Build history of the part. All positions in model axes, mm. Face numbers are marked on the shaded views. Give positions to 0.01 mm unless a question says otherwise; leave off trailing zeros. Loops run counter-clockwise (first coordinate to the right, second up) from the corner with the lowest first, then second, coordinate; pieces in that order, holes last. Notation, with made-up numbers: M 42.5,-13.5 L 77.5,-13.5 A28 ccw 77.5,15.5 Z; hole C 62.25,36.5 d9. An arc over 180 degrees is marked long. Answer in a Markdown table with one row per item. Add a question column.
```python
from build123d import *

# Parameters (mm, degrees)
SKETCH1_R           = 7
BOSS_EXTRUDE1_DEPTH = 10


with BuildPart() as part:
    # Sketch1 → Boss-Extrude1 (new body)
    with BuildSketch(Plane.XY):
        Polygon((-80, 104), (-30, 17.397459622), (0, 0), (100, 0), align=None)
        with Locations((2, 39)):
            Circle(SKETCH1_R, mode=Mode.SUBTRACT)
    extrude(amount=BOSS_EXTRUDE1_DEPTH)


solid = part.part
```
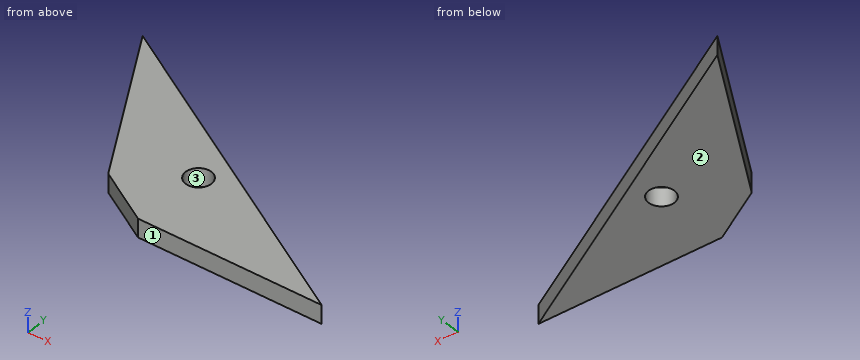
(1) Pull direction Y, two halves, no side cores. Call the marked faces 1, 2 and 3: +Y half, -Y half, draft (parallel to the pull), parting line (faces both ways), or undercut.
(2) Slice it at D-D, the plane x = 64. Give the cut face in (y, z).
(3) Pin check, flat tips, straight feed: pin 1 (3 mm diameter, centred on y = 26.5, z = 7, fed in from +X); pin 2 (1 mm diameter, centred on x = -33, z = 8.5, fed in from +Y); pin 3 (1 mm diameter, centred on x = 9.5, z = 7.5, fed in from +Y). Stop position of each tip, or through.
(4) Slice it at C-C, the plane z = 4.5. Give the cut face in (x, y).
(5) Slice it at A-A, the plane x = 2. Give the cut face in (y, z).
(6) Slice it at B-B, the plane y = 39. Give the cut face in (x, z).
(7) Wall check: line 1 (X direction, y = 33.5, z = 0.5); line 2 (Y direction, x = 2, z = 2); line 3 (X direction, y = 34.5, z = 6.5). Give the ranges that are in metal, low to high.
Solution:
| question | item | result |
|---|---|---|
| 1 | face 1 | -Y half |
| 1 | face 2 | draft |
| 1 | face 3 | undercut |
| 2 | outline | M 0,0 L 20.8,0 L 20.8,10 L 0,10 Z |
| 3 | pin 1 | x = 56.73 |
| 3 | pin 2 | y = 77.13 |
| 3 | pin 3 | y = 52.58 |
| 4 | outline | M -80,104 L -30,17.4 L 0,0 L 100,0 Z; hole C 2,39 d14 |
| 5 | outline | M 0,0 L 32,0 L 32,10 L 0,10 Z; M 46,0 L 56.62,0 L 56.62,10 L 46,10 Z |
| 6 | outline | M -42.47,0 L -5,0 L -5,10 L -42.47,10 Z; M 9,0 L 32.5,0 L 32.5,10 L 9,10 Z |
| 7 | line 1 | -39.3 to -2.33, 6.33 to 42.02 |
| 7 | line 2 | 0 to 32, 46 to 56.62 |
| 7 | line 3 | -39.87 to -3.36, 7.36 to 40.29 |
